Read the model definition and answer for the solid it produces. Units are mm, in the model's axes. A direction names the side the tool comes from. Coordinates: 2 decimals unless noted, no trailing zeros. Write each loop counter-clockwise with the first axis right and the second up, starting at its lowest first coordinate (ties: lowest second). Pieces come first, ordered by that corner, then holes. Notation, with made-up numbers: (68.5, -26.5) - (114.5, -26.5) arc R19 cw to (114.5, -18.5) - close; hole circle Ø1 at (28.5, 74.25). An arc over 180 degrees is marked (long way). Use a Markdown table: item, result.
from build123d import *

# Parameters (mm, degrees)
BASE_PLATE_SKETCH_W           = 78
BASE_PLATE_SKETCH_H           = 41
BASE_PLATE_SKETCH_R           = 5
BASE_PLATE_DEPTH              = 7
GUSSET_DEPTH                  = 7
UPRIGHT_WALL_DEPTH            = 7
KEYHOLE_FLANGE_SKETCH_W       = 70
KEYHOLE_FLANGE_SKETCH_H       = 38
KEYHOLE_MOUNTING_FLANGE_DEPTH = 7


with BuildPart() as part:
    # Base Plate Sketch → Base Plate (new body)
    with BuildSketch(Plane(origin=(0, 0, 0), x_dir=(1, 0, 0), z_dir=(0, 1, 0))):
        Rectangle(BASE_PLATE_SKETCH_W, BASE_PLATE_SKETCH_H)
        with Locations(Location((-19, -8.5, 0), (0, 0, 270))):
            Circle(BASE_PLATE_SKETCH_R, mode=Mode.SUBTRACT)
        with Locations(Location((19, -8.5, 0), (0, 0, 270))):
            Circle(BASE_PLATE_SKETCH_R, mode=Mode.SUBTRACT)
    extrude(amount=BASE_PLATE_DEPTH)

    # Gusset Sketch → Gusset (add)
    with BuildSketch(Plane.ZY.offset(39)):
        Polygon((-20.5, 7), (-20.5, 32), (20.5, 7), align=None)
    extrude(amount=-GUSSET_DEPTH)

    # Upright Wall Sketch → Upright Wall (add)
    with BuildSketch(Plane(origin=(0, 0, -20.5), x_dir=(-1, 0, 0), z_dir=(0, 0, -1))):
        Polygon((-39, 7), (-39, 33), (39, 69.371997336), (39, 7), align=None)
    extrude(amount=-UPRIGHT_WALL_DEPTH)

    # Keyhole Flange Sketch → Keyhole Mounting Flange (add)
    with BuildSketch(Plane(origin=(19.605374923, 42.043862201, 0), x_dir=(0.9063077870366493, -0.4226182617407009, 0), z_dir=(0.4226182617407009, 0.9063077870366493, 0))):
        with Locations((-19.663876622, 39.5)):
            Rectangle(KEYHOLE_FLANGE_SKETCH_W, KEYHOLE_FLANGE_SKETCH_H)
        with BuildLine():
            Line((-34.663876622, 42.5), (-12.72613437, 42.5))
            ThreePointArc((-12.72613437, 42.5), (4.336123378, 38.5), (-12.72613437, 34.5))
            Line((-12.72613437, 34.5), (-34.663876622, 34.5))
            ThreePointArc((-34.663876622, 34.5), (-38.663876622, 38.5), (-34.663876622, 42.5))
        make_face(mode=Mode.SUBTRACT)
    extrude(amount=-KEYHOLE_MOUNTING_FLANGE_DEPTH)


solid = part.part
(1) A cutting plane is placed at B-B, the plane z = -41. Write down the section's boundary in (x, y), and give its area (3 significant figures).
Report:
| item | result |
|---|---|
| outline | (-32.9, 58.8) - (-17.6, 51.67) - (-14.64, 58.01) - (-29.94, 65.15) - close; (20.26, 34.02) - (30.55, 29.22) - (33.5, 35.56) - (23.21, 40.36) - close |
| area | 198 mm² |
(2) A cutting plane is placed at D-D, the plane y = 19. Write down the section's boundary in (x, z), and give its area (3 significant figures).
Report:
| item | result |
|---|---|
| outline | (-39, -20.5) - (39, -20.5) - (39, -13.5) - (-32, -13.5) - (-32, 0.82) - (-39, 0.82) - close |
| area | 646 mm² |
(3) For faces 5 (the flat face through (32.046, 32.435, -39.234)), 6 (the flat face through (-32, 13, -4)), 7 (the flat face through (-31.395, 62.018, -39.234)), 8 (the flat face through (39, 5, -9)), determine the directions among +Z, -Z, +X, -X, +Y, -Y from which every point of the face is accessible in a straight line to the end or side of a thin tool.
Report:
| item | result |
|---|---|
| face 5 | -Z, +X, -Y |
| face 6 | +Z, +X, +Y |
| face 7 | -Z, -X, +Y |
| face 8 | +Z, -Z, +X, +Y, -Y |
(4) Straight lines are drawn through the part: L1, parallel to X at y = 5.75, z = 8.5; L2, parallel to Z at x = 14, y = 41; L3, parallel to Z at x = -26, y = 5.5. For each, find the intervals that lie inside material, in ascending order.
Report:
| item | result |
|---|---|
| L1 | x = -39 to -24, -14 to 14, 24 to 39 |
| L2 | z = -58.5 to -47.5, -29.5 to -13.5 |
| L3 | z = -20.5 to 20.5 |
(5) A cutting plane is placed at A-A, the plane z = 8.5. Write down the section's boundary in (x, y), and give its area (3 significant figures).
Report:
| item | result |
|---|---|
| outline | (-39, 0) - (-24, 0) - (-24, 7) - (-32, 7) - (-32, 14.32) - (-39, 14.32) - close; (-14, 0) - (14, 0) - (14, 7) - (-14, 7) - close; (24, 0) - (39, 0) - (39, 7) - (24, 7) - close |
| area | 457 mm² |
(6) Each of these flat-tipped pins is pushed along its axis until it touches: P1, Ø10, axis at x = -2.5, z = 1, coming from the +Y side; P2, Ø2, axis at x = -25, z = -44.5, coming from the -Y side; P3, Ø18.5, axis at x = 10.5, y = 29.5, coming from the +Z side; P4, Ø6, axis at x = 19, z = 8.5, coming from the +Y side. Where does it stop, or does it pass through?
Report:
| item | result |
|---|---|
| P1 | stops at y = 7 |
| P2 | stops at y = 54.65 |
| P3 | stops at z = -13.5 |
| P4 | passes through |
(7) A cutting plane is placed at C-C, the plane x = 1. Write down the section's boundary in (y, z), and give its area (3 significant figures).
Report:
| item | result |
|---|---|
| outline | (0, -20.5) - (43, -20.5) - (43, -34.5) - (50.72, -34.5) - (50.72, -13.5) - (7, -13.5) - (7, 20.5) - (0, 20.5) - close; (43, -58.5) - (50.72, -58.5) - (50.72, -42.5) - (43, -42.5) - close |
| area | 825 mm² |
(8) The mould has two halves that part along X. Classify faces 1 (the cylindrical face through (-23.436, 3.451, 10.807)), 2 (the flat face through (-1, 32, -13.5)), 3 (the cylindrical face through (14.564, 3.451, 10.807)), 4 (the flat face through (-1.619, 44.217, -43.988)): pulls with the +X half, pulls with the -X half, needs draft (parallel to the pull), parting line crosses it, or undercut.
Report:
| item | result |
|---|---|
| face 1 | undercut |
| face 2 | needs draft |
| face 3 | undercut |
| face 4 | pulls with the -X half |
